```python
from build123d import *


with BuildPart() as part:
    # 草图1 → 旋转1 (revolve)
    with BuildSketch(Plane(origin=(0, 0, 0), x_dir=(0, 0, -1), z_dir=(1, 0, 0)), mode=Mode.PRIVATE) as revolve_1_sk:
        Polygon((-19, 8), (-18, 7), (12, 7), (12, 9.9), (-19, 9.9), align=None)
    revolve(revolve_1_sk.sketch.rotate(Axis((0, 0, -12), (0, 0, 1)), 270), axis=Axis((0, 0, -12), (0, 0, 1)))

    # 草图2 → 切除-旋转1 (revolve, cut)
    with BuildSketch(Plane(origin=(0, 0, 0), x_dir=(0, 0, -1), z_dir=(1, 0, 0)), mode=Mode.PRIVATE) as cut_revolve_1_sk:
        Polygon((-15.5, 9.9), (-13.5, 9.9), (-13.879, 9.521), (-13.879, 7.379), (-13.5, 7), (-13.5, 0), (-15.5, 0), align=None)
    revolve(cut_revolve_1_sk.sketch.rotate(Axis((0, 0, 15.5), (0, 1, 0)), 180), axis=Axis((0, 0, 15.5), (0, 1, 0)), mode=Mode.SUBTRACT)


solid = part.part
```
The model under review builds one solid part; all positions refer to its coordinate system, in mm. A direction names the side the tool comes from. Round coordinates to 2 decimals unless told otherwise and drop trailing zeros. Write each loop counter-clockwise with the first axis right and the second up, starting at its lowest first coordinate (ties: lowest second). Pieces come first, ordered by that corner, then holes.
(1) Wall thickness on L1, parallel to X at y = 0.25, z = -6; L2, parallel to X at y = -3.75, z = 17.5: over which ranges is each line inside the solid? List them lowest first.
(2) Insertion check: pin 1 (3 mm diameter, centred on y = -3, z = 3, fed in from -X); pin 2 (11 mm diameter, centred on x = 0, y = 0, fed in from +Z); pin 3 (3 mm diameter, centred on x = 6.5, z = 10, fed in from +Y); pin 4 (2 mm diameter, centred on y = 6, z = 15, fed in from -X). Each pin has a flat end and moves straight along its axis. Give the tip position at first contact, or say it passes through.
(3) We need section A-A on y = 0. Give the boundary of the cut face in (x, z), and give its area (3 significant figures).
(4) We need section B-B on z = 6. Give the boundary of the cut face in (x, y), and give its area (3 significant figures).
(5) Machinability: for faces 4 (the cylindrical face through (-0.621, 8.435, 16.997)), 5 (the flat face through (-2, 7, -12)), which of the approach directions +Z, -Z, +X, -X, +Y, -Y give a long, thin tool a straight path to every point of the face, cutting with its end or side? Answer none if there is none.
(6) Mouldability with a two-part tool opening along Y and no side actions: class faces 1 (the cylindrical face through (9.443, 2.974, 3.717)), 2 (the cylindrical face through (-1.517, -6.834, 2.79)), 3 (the flat face through (-3.7, -7.3, 19)) as +Y half, -Y half, draft (parallel to the pull), parting line (faces both ways), or undercut.
(7) We need section C-C on z = 15.5. Give the boundary of the cut face in (x, y).
Findings below:
1. L1: x = -9.9 to -7, 7 to 9.9
1. L2: x = -9.16 to -5.91, 5.91 to 9.16
2. pin 1: stops at x = -9.79
2. pin 2: passes through
2. pin 3: stops at y = 8.54
2. pin 4: stops at x = -8.54
3. outline: (-9.9, -12) - (-7, -12) - (-7, 18) - (-8, 19) - (-9.9, 19) - close; (7, -12) - (9.9, -12) - (9.9, 19) - (8, 19) - (7, 18) - close
3. area: 179 mm2
4. outline: circle Ø19.8 at (0, 0); hole circle Ø14 at (0, 0)
4. area: 154 mm2
5. face 4: +Y
5. face 5: -Z, +X, -X, +Y, -Y
6. face 1: parting line
6. face 2: undercut
6. face 3: draft
7. outline: (-2, 6.71) - (-2, 7) - (-1.62, 7.38) - (-1.62, 9.52) - (-1.83, 9.73) arc R9.9 ccw (long way) to (1.83, 9.73) - (1.62, 9.52) - (1.62, 7.38) - (2, 7) - (2, 6.71) arc R7 cw (long way) to start
